Geometry check sheet. Reference: drawing and pictorial views, mm from the part's lowest x, y, z. Give positions to 0.01 mm unless a question says otherwise; leave off trailing zeros. Write each loop counter-clockwise with the first axis right and the second up, starting at its lowest first coordinate (ties: lowest second). Pieces come first, ordered by that corner, then holes.
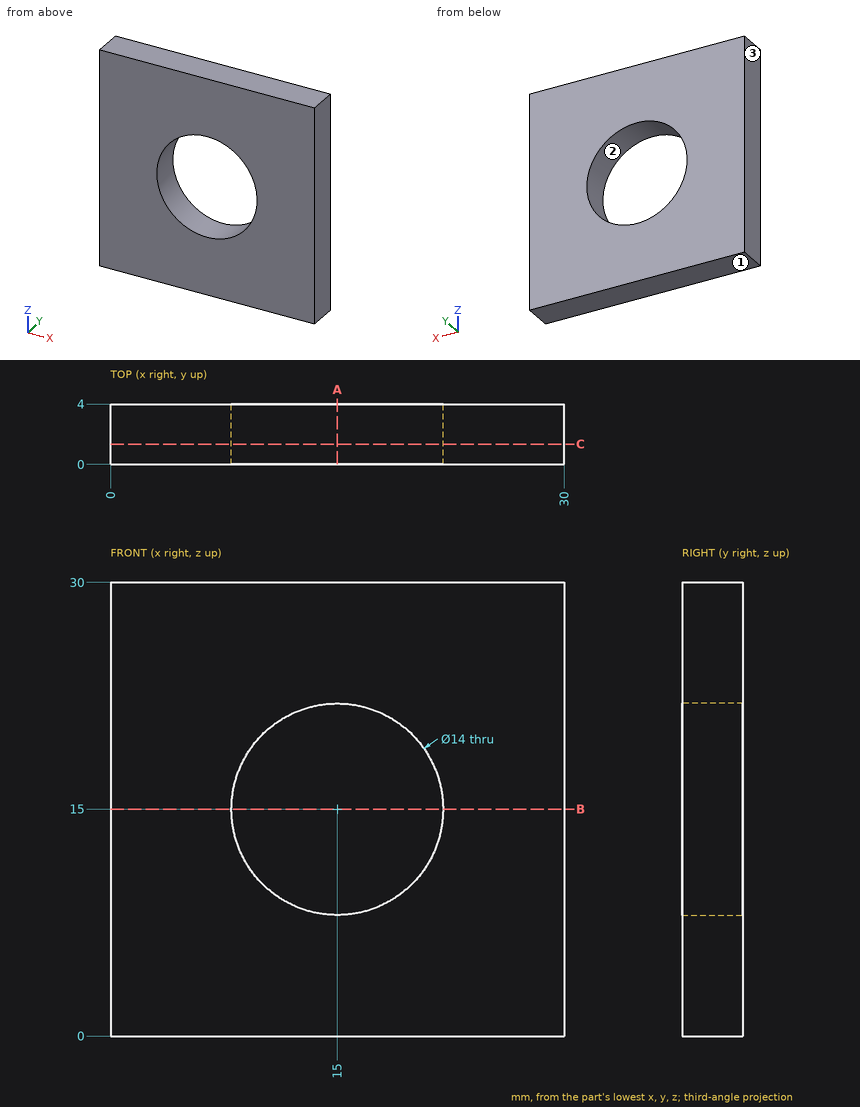
Item 1: Release check for a two-part mould opening along Z. For the marked faces 1, 2 and 3 record: released by +Z, released by -Z, zero draft, split by the parting line, or undercut.
Answer key:
face 1: released by -Z
face 2: undercut
face 3: zero draft
Item 2: Sectioned sample at C-C on y = 1.35. Record the cut outline in (x, z), then the cut area to 3 significant figures.
Answer key:
outline: (0, 0) - (30, 0) - (30, 30) - (0, 30) - close; hole circle Ø14 at (15, 15)
area: 746 mm2
Item 3: Sectioned sample at B-B on z = 15. Record the cut outline in (x, y), then the cut area to 3 significant figures.
Answer key:
outline: (0, 0) - (8, 0) - (8, 4) - (0, 4) - close; (22, 0) - (30, 0) - (30, 4) - (22, 4) - close
area: 64.0 mm2
Item 4: Depth check by flat-ended pin: pin 1 (8 mm diameter, centred on x = 17.5, z = 6, fed in from -Y). Enter the tip coordinate at first touch or a pass-through.
Answer key:
pin 1: stops at y = 0
Item 5: Sectioned sample at A-A on x = 15. Record the cut outline in (y, z), then the cut area to 3 significant figures.
Answer key:
outline: (0, 0) - (4, 0) - (4, 8) - (0, 8) - close; (0, 22) - (4, 22) - (4, 30) - (0, 30) - close
area: 64.0 mm2
Item 6: Scan lines: line 1 along Z through (x, y) = (15.25, 1.5); line 2 along Z through (x, y) = (12.75, 1.65). Record each from-to range of solid material in increasing order.
Answer key:
line 1: z = 0 to 8, 22 to 30
line 2: z = 0 to 8.37, 21.63 to 30
